Read the model definition and answer for the solid it produces. Units are mm, in the model's axes. A direction names the side the tool comes from. Coordinates: 2 decimals unless noted, no trailing zeros. Write each loop counter-clockwise with the first axis right and the second up, starting at its lowest first coordinate (ties: lowest second). Pieces come first, ordered by that corner, then holes. Notation, with made-up numbers: (77, -20) - (113, -20) arc R29 cw to (113, 8) - close; hole circle Ø6 at (13.5, 20.25). An arc over 180 degrees is marked (long way). Use a Markdown table: item, result.
from build123d import *

# Parameters (mm, degrees)
BLOCK_PROFILE_SKETCH_W    = 45
BLOCK_PROFILE_SKETCH_H    = 50
BLOCK_PROFILE_SKETCH_W_2  = 15
BLOCK_PROFILE_SKETCH_H_2  = 15
BLOCK_BODY_90MM_DEPTH     = 45
CENTER_POCKET_SKETCH_W    = 70
CENTER_POCKET_SKETCH_H    = 35
CENTER_POCKET_35X70_DEPTH = 40
POCKET_PAD_SKETCH_R       = 10
POCKET_PAD_5MM_DEPTH      = 5
SIDE_HOLE_REACH           = 64.249
SIDE_HOLE_SKETCH_R        = 10
SUPPORT_RIB_8MM_REACH     = 58.181
SUPPORT_RIB_SKETCH_WALL_W = 144.774837922
SUPPORT_RIB_SKETCH_WALL_H = 8


with BuildPart() as part:
    # Block Profile Sketch → Block Body 90mm (new, symmetric)
    with BuildSketch(Plane(origin=(0, 0, 0), x_dir=(0, 0, -1), z_dir=(1, 0, 0))):
        Rectangle(BLOCK_PROFILE_SKETCH_W, BLOCK_PROFILE_SKETCH_H)
        with Locations((5, 2.5)):
            Rectangle(BLOCK_PROFILE_SKETCH_W_2, BLOCK_PROFILE_SKETCH_H_2, mode=Mode.SUBTRACT)
    extrude(amount=BLOCK_BODY_90MM_DEPTH, both=True)

    # Center Pocket Sketch → Center Pocket 35x70 (cut)
    with BuildSketch(Plane(origin=(0, 25, 0), x_dir=(1, 0, 0), z_dir=(0, 1, 0))):
        with Locations((0, 5)):
            Rectangle(CENTER_POCKET_SKETCH_W, CENTER_POCKET_SKETCH_H)
    extrude(amount=-CENTER_POCKET_35X70_DEPTH, mode=Mode.SUBTRACT)

    # Pocket Pad Sketch → Pocket Pad 5mm (add)
    with BuildSketch(Plane(origin=(0, 0, 12.5), x_dir=(-1, 0, 0), z_dir=(0, 0, -1))):
        with BuildLine():
            Line((20, 10), (35, 10))
            Line((35, 10), (35, 25))
            Line((35, 25), (-35, 25))
            Line((-35, 25), (-35, 10))
            Line((-35, 10), (-20, 10))
            ThreePointArc((-20, 10), (0, -10), (20, 10))
        make_face()
        with Locations((0, 10)):
            Circle(POCKET_PAD_SKETCH_R, mode=Mode.SUBTRACT)
    extrude(amount=POCKET_PAD_5MM_DEPTH)

    # Side Hole Sketch → Side Hole (cut, up to next)
    with BuildSketch(Plane(origin=(0, 0, 12.5), x_dir=(-1, 0, 0), z_dir=(0, 0, -1)), mode=Mode.PRIVATE) as side_hole_sk1:
        with Locations((0, 10)):
            Circle(SIDE_HOLE_SKETCH_R)
    side_hole_tool1 = extrude(side_hole_sk1.sketch, amount=-SIDE_HOLE_REACH, mode=Mode.PRIVATE) & part.part
    add(side_hole_tool1.solids().sort_by_distance((0, 10, 12.5))[0], mode=Mode.SUBTRACT)

    # Support Rib Sketch wall → Support Rib 8mm (add, up to next)
    with BuildSketch(Plane(origin=(0, -12.5, -7.5), x_dir=(0, -0.164398987305, -0.986393923832), z_dir=(0, 0.986393923832, -0.164398987305)), mode=Mode.PRIVATE) as support_rib_8mm_sk1:
        Rectangle(SUPPORT_RIB_SKETCH_WALL_W, SUPPORT_RIB_SKETCH_WALL_H)
    support_rib_8mm_tool1 = extrude(support_rib_8mm_sk1.sketch, amount=-SUPPORT_RIB_8MM_REACH, mode=Mode.PRIVATE) - part.part
    add(support_rib_8mm_tool1.solids().sort_by_distance((0, -12.5, -7.5))[0])


solid = part.part
(1) A cutting plane is placed at A-A, the plane x = -6. Write down the section's boundary in (y, z).
Report:
| item | result |
|---|---|
| outline | (-25, -22.5) - (-15, -22.5) - (-15, 12.5) - (-9.08, 12.5) - (-9.08, 7.5) - (2, 7.5) - (2, 22.5) - (-25, 22.5) - close; (18, 7.5) - (25, 7.5) - (25, 22.5) - (18, 22.5) - close |
(2) The mould has two halves that part along X. Classify faces 1 (the flat face through (40, 2, -12.5)), 2 (the cylindrical face through (14.297, -3.986, 10.035)), 3 (the flat face through (28, 10, 10)): pulls with the +X half, pulls with the -X half, needs draft (parallel to the pull), parting line crosses it, or undercut.
Report:
| item | result |
|---|---|
| face 1 | needs draft |
| face 2 | undercut |
| face 3 | undercut |
(3) For faces 4 (the flat face through (-40, -5, -5)), 5 (the flat face through (1, -25, 0)), 6 (the flat face through (-23, -5, 12.5)), determine the directions among +Z, -Z, +X, -X, +Y, -Y from which every point of the face is accessible in a straight line to the end or side of a thin tool.
Report:
| item | result |
|---|---|
| face 4 | +X, -X |
| face 5 | +Z, -Z, +X, -X, -Y |
| face 6 | -Z |
(4) A cutting plane is placed at C-C, the plane y = 17. Write down the section's boundary in (x, z).
Report:
| item | result |
|---|---|
| outline | (-45, -22.5) - (-35, -22.5) - (-35, 7.5) - (-7.14, 7.5) - (-7.14, 22.5) - (-45, 22.5) - close; (7.14, 7.5) - (35, 7.5) - (35, -22.5) - (45, -22.5) - (45, 22.5) - (7.14, 22.5) - close |
(5) A cutting plane is placed at D-D, the plane z = 15.5. Write down the section's boundary in (x, y).
Report:
| item | result |
|---|---|
| outline | (-45, -25) - (45, -25) - (45, 25) - (-45, 25) - close; hole circle Ø20 at (0, 10) |
(6) Straight lines are drawn through the part: L1, parallel to Y at x = -38.5, z = 2; L2, parallel to Y at x = 0, z = 20; L3, parallel to Z at x = 41.5, y = -0.5. For each, find the intervals that lie inside material, in ascending order.
Report:
| item | result |
|---|---|
| L1 | y = -25 to -5, 10 to 25 |
| L2 | y = -25 to 0, 20 to 25 |
| L3 | z = -22.5 to -12.5, 2.5 to 22.5 |
(7) Each of these flat-tipped pins is pushed along its axis until it touches: P1, Ø12, axis at x = -26.5, z = -17, coming from the +Y side; P2, Ø7.5, axis at x = -22, y = -4.5, coming from the -Z side; P3, Ø12, axis at x = 1, z = 4, coming from the +Y side; P4, Ø20, axis at x = 14.5, y = 2.5, coming from the -Z side. Where does it stop, or does it pass through?
Report:
| item | result |
|---|---|
| P1 | stops at y = -15 |
| P2 | stops at z = 12.5 |
| P3 | stops at y = 25 |
| P4 | stops at z = 7.5 |
(8) A cutting plane is placed at B-B, the plane z = -11.5. Write down the section's boundary in (x, y).
Report:
| item | result |
|---|---|
| outline | (-45, -25) - (45, -25) - (45, -5) - (35, -5) - (35, -15) - (4, -15) - (4, -13.17) - (-4, -13.17) - (-4, -15) - (-35, -15) - (-35, -5) - (-45, -5) - close; (-45, 10) - (-35, 10) - (-35, 25) - (-45, 25) - close; (35, 10) - (45, 10) - (45, 25) - (35, 25) - close |
